Could you check a few things on this drawing? It's one solid part, dimensions in mm from its lowest x, y, z. Coordinates: 2 decimals unless noted, no trailing zeros. Order: outer loops, then holes, each group sorted by start corner. A loop starts at its lowest first (then second) coordinate and runs counter-clockwise, first axis right, second up. Notation, with made-up numbers: (0.5, 80.25) - (44.5, 80.25) arc R16 ccw to (44.5, 89.25) - close; hole circle Ø2 at (-37, 83.25). An arc over 180 degrees is marked (long way). Answer in a Markdown table with one row per item. Add a question column.
Item 1: I want a section at D-D (y = 6). Please give me the cut outline in (x, z).
Item 2: I want a section at B-B (y = 85). Please give me the cut outline in (x, z), plus the area to 3 significant figures.
Item 3: I want a section at C-C (z = 4.5). Please give me the cut outline in (x, y), plus the area to 3 significant figures.
Item 4: I want a section at A-A (x = 15). Please give me the cut outline in (y, z), plus the area to 3 significant figures.
Item 5: Will these pins go through, and if not, where does the flat tip stop? pin 1 Ø1.5 at (x, y) = (98, 48) entering from -Z; pin 2 Ø8 at (x, y) = (95, 85) entering from +Z.
Item 6: If I drill on line 1 along Y through (x, z) = (15, 5); line 2 along X through (y, z) = (81, 2.5); line 3 along Y through (x, z) = (93, 13), over which ranges is the centre line in solid material (lowest first)? Write a range as from..to.
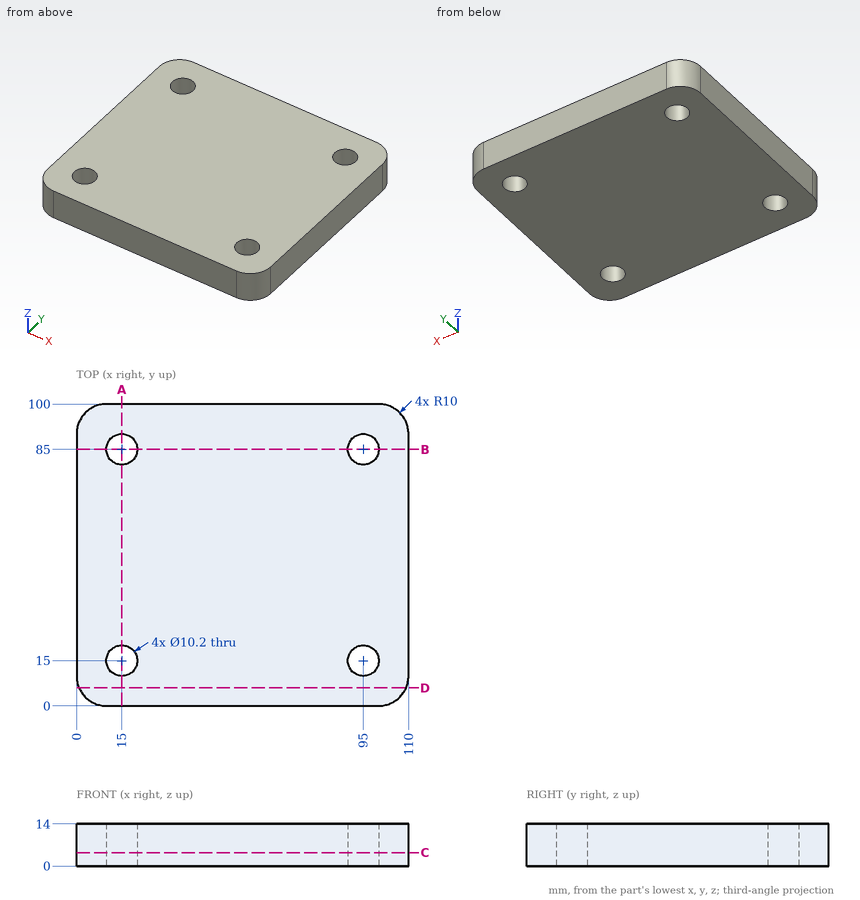
Values follow:
| question | item | result |
|---|---|---|
| 1 | outline | (0.83, 0) - (109.17, 0) - (109.17, 14) - (0.83, 14) - close |
| 2 | outline | (0, 0) - (9.9, 0) - (9.9, 14) - (0, 14) - close; (20.1, 0) - (89.9, 0) - (89.9, 14) - (20.1, 14) - close; (100.1, 0) - (110, 0) - (110, 14) - (100.1, 14) - close |
| 2 | area | 1,250 mm^2 |
| 3 | outline | (0, 10) arc R10 ccw to (10, 0) - (100, 0) arc R10 ccw to (110, 10) - (110, 90) arc R10 ccw to (100, 100) - (10, 100) arc R10 ccw to (0, 90) - close; hole circle Ø10.2 at (15, 15); hole circle Ø10.2 at (15, 85); hole circle Ø10.2 at (95, 15); hole circle Ø10.2 at (95, 85) |
| 3 | area | 10,600 mm^2 |
| 4 | outline | (0, 0) - (9.9, 0) - (9.9, 14) - (0, 14) - close; (20.1, 0) - (79.9, 0) - (79.9, 14) - (20.1, 14) - close; (90.1, 0) - (100, 0) - (100, 14) - (90.1, 14) - close |
| 4 | area | 1,110 mm^2 |
| 5 | pin 1 | stops at z = 0 |
| 5 | pin 2 | passes through |
| 6 | line 1 | y = 0..9.9, 20.1..79.9, 90.1..100 |
| 6 | line 2 | x = 0..11.84, 18.16..91.84, 98.16..110 |
| 6 | line 3 | y = 0..10.31, 19.69..80.31, 89.69..100 |
